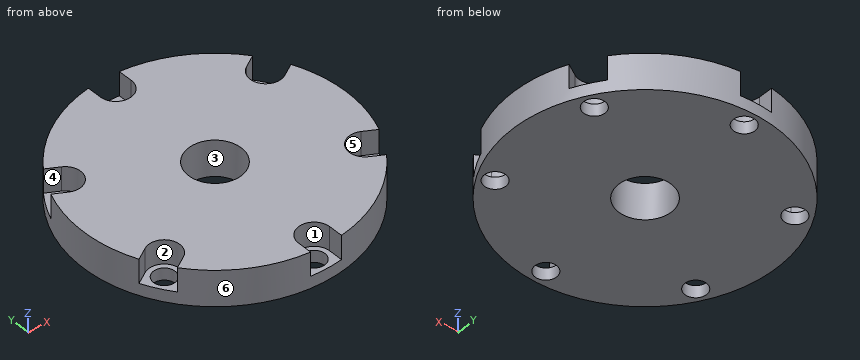
from build123d import *

# Parameters (mm, degrees)
SKETCH1_R           = 110
SKETCH1_R_2         = 9
SKETCH1_R_3         = 22
BOSS_EXTRUDE1_DEPTH = 30
CUT_EXTRUDE1_DEPTH  = 20


with BuildPart() as part:
    # Sketch1 → Boss-Extrude1 (new body)
    with BuildSketch(Plane.XY):
        Circle(SKETCH1_R)
        with Locations((0, 97.5)):
            Circle(SKETCH1_R_2, mode=Mode.SUBTRACT)
        with Locations((84.437476869, 48.75)):
            Circle(SKETCH1_R_2, mode=Mode.SUBTRACT)
        with Locations((84.437476869, -48.75)):
            Circle(SKETCH1_R_2, mode=Mode.SUBTRACT)
        with Locations((0, -97.5)):
            Circle(SKETCH1_R_2, mode=Mode.SUBTRACT)
        with Locations((-84.437476869, -48.75)):
            Circle(SKETCH1_R_2, mode=Mode.SUBTRACT)
        with Locations((-84.437476869, 48.75)):
            Circle(SKETCH1_R_2, mode=Mode.SUBTRACT)
        Circle(SKETCH1_R_3, mode=Mode.SUBTRACT)
    extrude(amount=BOSS_EXTRUDE1_DEPTH)

    # Sketch2 → Cut-Extrude1 (cut)
    with BuildSketch(Plane.XY.offset(30)):
        with BuildLine():
            Line((-13, 97.5), (-13, 114.531439902))
            Line((-13, 114.531439902), (13, 114.531439902))
            Line((13, 114.531439902), (13, 97.5))
            ThreePointArc((13, 97.5), (0, 84.5), (-13, 97.5))
        make_face()
        with BuildLine():
            Line((105.687136487, 46.007389702), (90.937476869, 37.491669751))
            ThreePointArc((90.937476869, 37.491669751), (73.17914662, 42.25), (77.937476869, 60.008330249))
            Line((77.937476869, 60.008330249), (92.687136487, 68.5240502))
            Line((92.687136487, 68.5240502), (105.687136487, 46.007389702))
        make_face()
        with BuildLine():
            Line((92.687136487, -68.5240502), (77.937476869, -60.008330249))
            ThreePointArc((77.937476869, -60.008330249), (73.17914662, -42.25), (90.937476869, -37.491669751))
            Line((90.937476869, -37.491669751), (105.687136487, -46.007389702))
            Line((105.687136487, -46.007389702), (92.687136487, -68.5240502))
        make_face()
        with BuildLine():
            Line((-13, -114.531439902), (-13, -97.5))
            ThreePointArc((-13, -97.5), (0, -84.5), (13, -97.5))
            Line((13, -97.5), (13, -114.531439902))
            Line((13, -114.531439902), (-13, -114.531439902))
        make_face()
        with BuildLine():
            Line((-105.687136487, -46.007389702), (-90.937476869, -37.491669751))
            ThreePointArc((-90.937476869, -37.491669751), (-73.17914662, -42.25), (-77.937476869, -60.008330249))
            Line((-77.937476869, -60.008330249), (-92.687136487, -68.5240502))
            Line((-92.687136487, -68.5240502), (-105.687136487, -46.007389702))
        make_face()
        with BuildLine():
            Line((-92.687136487, 68.5240502), (-77.937476869, 60.008330249))
            ThreePointArc((-77.937476869, 60.008330249), (-73.17914662, 42.25), (-90.937476869, 37.491669751))
            Line((-90.937476869, 37.491669751), (-105.687136487, 46.007389702))
            Line((-105.687136487, 46.007389702), (-92.687136487, 68.5240502))
        make_face()
    extrude(amount=-CUT_EXTRUDE1_DEPTH, mode=Mode.SUBTRACT)


solid = part.part
For this review, take the finished solid that the model builds, in its own axes (mm). Face numbers are marked on the shaded views. A direction names the side the tool comes from. Round coordinates to 2 decimals unless told otherwise and drop trailing zeros. Write each loop counter-clockwise with the first axis right and the second up, starting at its lowest first coordinate (ties: lowest second). Pieces come first, ordered by that corner, then holes. Notation, with made-up numbers: (37.25, 39.25) - (84.25, 39.25) arc R27 cw to (84.25, 74.25) - close; hole circle Ø9 at (19, 26). An arc over 180 degrees is marked (long way). Write item = value, one per line. Start each with the question number.
1. For the marked faces 1, 2 and 3, list the 3-axis set-ups (+Z, -Z, +X, -X, +Y, -Y) from which the entire face can be reached by the end or side of a thin tool; tool diameter is ignored.
2. For pin 1 Ø16 at (x, y) = (-84.44, -48.75) entering from +Z; pin 2 Ø9 at (x, y) = (-91, -44) entering from +Z; pin 3 Ø4 at (y, z) = (-7.5, 3.5) entering from -X; pin 4 Ø5 at (y, z) = (-25.5, 8) entering from -X, all flat-tipped, find the tip position at first contact; note any pin that passes through.
3. Consider section A-A on x = 0. State the section outline as (y, z) points.
4. Consider section C-C on y = 3. State the section outline as (x, z) points, plus the area to 3 significant figures.
5. Consider section B-B on z = 20.5. State the section outline as (x, y) points, plus the area to 3 significant figures.
6. Wall thickness on L1, parallel to Y at x = 0, z = 7; L2, parallel to Y at x = -78.5, z = 15.75; L3, parallel to X at y = 39, z = 25: over which ranges is each line inside the solid? List them lowest first.
7. Draft analysis for pull direction X (two halves, no side actions). For the marked faces 4, 5 and 6, state which applies: released by +X, released by -X, zero draft, split by the parting line, or undercut.
8. Consider section D-D on z = 6.75. State the section outline as (x, y) points.
Evaluation:
q1.face_1 = +Z, -Y
q1.face_2 = +Z
q1.face_3 = +Z, -Z
q2.pin_1 = through
q2.pin_2 = 10
q2.pin_3 = -109.86
q2.pin_4 = -107.57
q3.outline = (-110, 0) - (-106.5, 0) - (-106.5, 10) - (-110, 10) - close; (-88.5, 0) - (-22, 0) - (-22, 30) - (-84.5, 30) - (-84.5, 10) - (-88.5, 10) - close; (22, 0) - (88.5, 0) - (88.5, 10) - (84.5, 10) - (84.5, 30) - (22, 30) - close; (106.5, 0) - (110, 0) - (110, 10) - (106.5, 10) - close
q4.outline = (-109.96, 0) - (-21.79, 0) - (-21.79, 30) - (-109.96, 30) - close; (21.79, 0) - (109.96, 0) - (109.96, 30) - (21.79, 30) - close
q4.area = 5,290 mm2
q5.outline = (-101.1, -43.36) - (-90.94, -37.49) arc R13 cw to (-77.94, -60.01) - (-88.1, -65.87) arc R110 ccw to (-13, -109.23) - (-13, -97.5) arc R13 cw to (13, -97.5) - (13, -109.23) arc R110 ccw to (88.1, -65.87) - (77.94, -60.01) arc R13 cw to (90.94, -37.49) - (101.1, -43.36) arc R110 ccw to (101.1, 43.36) - (90.94, 37.49) arc R13 cw to (77.94, 60.01) - (88.1, 65.87) arc R110 ccw to (13, 109.23) - (13, 97.5) arc R13 cw to (-13, 97.5) - (-13, 109.23) arc R110 ccw to (-88.1, 65.87) - (-77.94, 60.01) arc R13 cw to (-90.94, 37.49) - (-101.1, 43.36) arc R110 ccw to start; hole circle Ø44 at (0, 0)
q5.area = 33,000 mm2
q6.L1 = -110 to -106.5, -88.5 to -22, 22 to 88.5, 106.5 to 110
q6.L2 = -77.06 to -60.33, -37.19 to 37.19, 60.33 to 77.06
q6.L3 = -102.85 to -93.55, -75.84 to 75.84, 93.55 to 102.85
q7.face_4 = released by -X
q7.face_5 = undercut
q7.face_6 = split by the parting line
q8.outline = circle Ø220 at (0, 0); hole circle Ø18 at (-84.44, -48.75); hole circle Ø18 at (-84.44, 48.75); hole circle Ø44 at (0, 0); hole circle Ø18 at (0, -97.5); hole circle Ø18 at (0, 97.5); hole circle Ø18 at (84.44, -48.75); hole circle Ø18 at (84.44, 48.75)
